The model under review builds one solid part; all positions refer to its coordinate system, in mm. Face numbers are marked on the shaded views. A direction names the side the tool comes from. Round coordinates to 2 decimals unless told otherwise and drop trailing zeros. Write each loop counter-clockwise with the first axis right and the second up, starting at its lowest first coordinate (ties: lowest second). Pieces come first, ordered by that corner, then holes. Notation, with made-up numbers: (11, 31) - (57, 31) arc R22 ccw to (57, 58) - close; hole circle Ø3 at (41.5, 37). An arc over 180 degrees is marked (long way). Write each question's results on one line, items separated by ' | '.
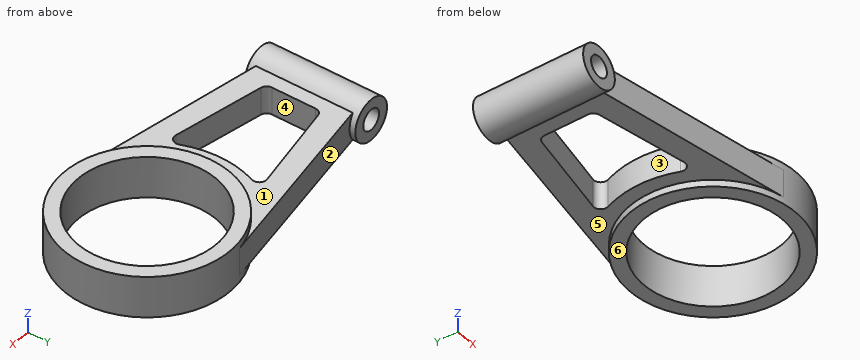
```python
from build123d import *

# Parameters (mm, degrees)
BIG_END_RING_SKETCH_R       = 60
BIG_END_RING_SKETCH_R_2     = 50
BIG_END_RING_120_DEPTH      = 15
SMALL_END_BOSS_SKETCH_R     = 15
SMALL_END_BOSS_SKETCH_R_2   = 7.5
SMALL_END_BOSS_30_DEPTH     = 40
CONNECTING_WEB_DEPTH        = 10
WEB_LIGHTENING_WINDOW_DEPTH = 52.5


with BuildPart() as part:
    # Big End Ring Sketch → Big End Ring Ø120 (new, symmetric)
    with BuildSketch(Plane.XY):
        Circle(BIG_END_RING_SKETCH_R)
        Circle(BIG_END_RING_SKETCH_R_2, mode=Mode.SUBTRACT)
    extrude(amount=BIG_END_RING_120_DEPTH, both=True)



with BuildPart() as body_2:
    # Small End Boss Sketch → Small End Boss Ø30 (new, symmetric)
    with BuildSketch(Plane(origin=(0, 0, 0), x_dir=(1, 0, 0), z_dir=(0, 1, 0))):
        with Locations(Location((-160, 0, 0), (0, 0, 270))):
            Circle(SMALL_END_BOSS_SKETCH_R)
        with Locations(Location((-160, 0, 0), (0, 0, 270))):
            Circle(SMALL_END_BOSS_SKETCH_R_2, mode=Mode.SUBTRACT)
    extrude(amount=SMALL_END_BOSS_30_DEPTH, both=True)


with BuildPart() as part_1:
    add(part.part)

    add(body_2.part)  # Connecting Web merges body 2
    # Web Profile Sketch → Connecting Web (add, symmetric)
    with BuildSketch(Plane.XY):
        with BuildLine():
            Line((-10.212938139, 59.12441031), (-149.873192049, 35))
            Line((-149.873192049, 35), (-149.873192049, -35))
            Line((-149.873192049, -35), (-10.212938139, -59.12441031))
            ThreePointArc((-10.212938139, -59.12441031), (-60, 0), (-10.212938139, 59.12441031))
        make_face()
    extrude(amount=CONNECTING_WEB_DEPTH, both=True)

    # Web Window Sketch → Web Lightening Window (cut, symmetric)
    with BuildSketch(Plane.XY.offset(10)):
        with BuildLine():
            Line((-138.819660113, 15.867947938), (-138.819660113, -15.867947938))
            ThreePointArc((-138.819660113, -15.867947938), (-137.673856674, -19.053096108), (-134.761592567, -20.778422788))
            Line((-134.761592567, -20.778422788), (-70.43555138, -33.117511712))
            ThreePointArc((-70.43555138, -33.117511712), (-65.629029038, -31.379566609), (-64.860710998, -26.326567738))
            ThreePointArc((-64.860710998, -26.326567738), (-70, 0), (-64.860710998, 26.326567738))
            ThreePointArc((-64.860710998, 26.326567738), (-65.629029038, 31.379566609), (-70.43555138, 33.117511712))
            Line((-70.43555138, 33.117511712), (-134.761592567, 20.778422788))
            ThreePointArc((-134.761592567, 20.778422788), (-137.673856674, 19.053096108), (-138.819660113, 15.867947938))
        make_face()
    extrude(amount=WEB_LIGHTENING_WINDOW_DEPTH, both=True, mode=Mode.SUBTRACT)


solid = part_1.part
```
Q1. Insertion check: P1, Ø5, axis at y = 12.5, z = 7.5, coming from the -X side; P2, Ø3, axis at y = -31.5, z = 7.5, coming from the -X side; P3, Ø4, axis at x = -69, z = 1.5, coming from the +Y side. Each pin has a flat end and moves straight along its axis. Give the tip position at first contact, or say it passes through.
Evaluation:
P1: stops at x = -174.14 | P2: stops at x = -173.75 | P3: stops at y = 49.32
Q2. The part is to be moulded in two halves that separate along Y. For the marked faces 1, 2 and 3, say which applies: released by +Y, released by -Y, zero draft, split by the parting line, or undercut.
Evaluation:
face 1: zero draft | face 2: released by +Y | face 3: undercut
Q3. We need section B-B (y = 0). State the section outline as (x, z) points.
Evaluation:
outline: (-148.82, -10) - (-138.82, -10) - (-138.82, 10) - (-148.82, 10) arc R15 ccw (long way) to start; (-70, -10) - (-60, -10) - (-60, -15) - (-50, -15) - (-50, 15) - (-60, 15) - (-60, 10) - (-70, 10) - close; (50, -15) - (60, -15) - (60, 15) - (50, 15) - close; hole circle Ø15 at (-160, 0)
Q4. We need section C-C (z = 0). State the section outline as (x, y) points.
Evaluation:
outline: (-175, -40) - (-167.5, -40) - (-167.5, 40) - (-175, 40) - close; (-152.5, -40) - (-145, -40) - (-145, -35.84) - (-10.21, -59.12) arc R60 ccw (long way) to (-10.21, 59.12) - (-145, 35.84) - (-145, 40) - (-152.5, 40) - close; hole (-138.82, -15.87) arc R5 ccw to (-134.76, -20.78) - (-70.44, -33.12) arc R5 ccw to (-64.86, -26.33) arc R70 cw to (-64.86, 26.33) arc R5 ccw to (-70.44, 33.12) - (-134.76, 20.78) arc R5 ccw to (-138.82, 15.87) - close; hole circle Ø100 at (0, 0)
Q5. Tool access review of the marked faces 4, 5 and 6: name each direction out of +Z, -Z, +X, -X, +Y, -Y from which nothing blocks a thin tool from reaching the whole face with its end or side.
Evaluation:
face 4: +Z, -Z | face 5: -Z | face 6: -Z, +X, -X, +Y, -Y
Q6. We need section D-D (x = 0). State the section outline as (y, z) points.
Evaluation:
outline: (-60, -15) - (-50, -15) - (-50, 15) - (-60, 15) - close; (50, -15) - (60, -15) - (60, 15) - (50, 15) - close
Q7. For probe 1 along X at (y, z) = (-9, 0); probe 2 along X at (y, z) = (-6.5, 0); probe 3 along X at (y, z) = (31.5, -10.25), list the stretches that pass through material, from the lowest coordinate up.
Evaluation:
probe 1: x = -175 to -167.5, -152.5 to -138.82, -69.42 to -49.18, 49.18 to 59.32 | probe 2: x = -175 to -167.5, -152.5 to -138.82, -69.7 to -49.58, 49.58 to 59.65 | probe 3: x = -170.95 to -149.05, -51.07 to -38.83, 38.83 to 51.07
Q8. We need section A-A (x = -160). State the section outline as (y, z) points.
Evaluation:
outline: (-40, -15) - (40, -15) - (40, -7.5) - (-40, -7.5) - close; (-40, 7.5) - (40, 7.5) - (40, 15) - (-40, 15) - close
